The model under review builds one solid part; all positions refer to its coordinate system, in mm. Round coordinates to 2 decimals unless told otherwise and drop trailing zeros. Order: outer loops, then holes, each group sorted by start corner. A loop starts at its lowest first (then second) coordinate and runs counter-clockwise, first axis right, second up. Notation, with made-up numbers: (36, -4.75) -> (68, -4.75) arc R24 cw to (68, 34.25) -> close; hole circle Ø3 at (11, 23). An arc over 180 degrees is marked (long way). Put each result on its own line as item: value. Start each with the question number.
from build123d import *

# Parameters (mm, degrees)
SKETCH_1_W      = 30
SKETCH_1_H      = 60
EXTRUDE_1_DEPTH = 209
SHELL_1_T       = -2


with BuildPart() as part:
    # 草图1 → 凸台-拉伸1 (new, symmetric)
    with BuildSketch(Plane.XY):
        Rectangle(SKETCH_1_W, SKETCH_1_H)
    extrude(amount=EXTRUDE_1_DEPTH, both=True)

    # 抽壳1
    shell_1_openings = [part.faces().sort_by_distance(p)[0] for p in [
        (0, 0, 209),
        (0, 0, -209),
        (0, 30, 0),
    ]]
    offset(amount=SHELL_1_T, openings=shell_1_openings, kind=Kind.INTERSECTION)


solid = part.part
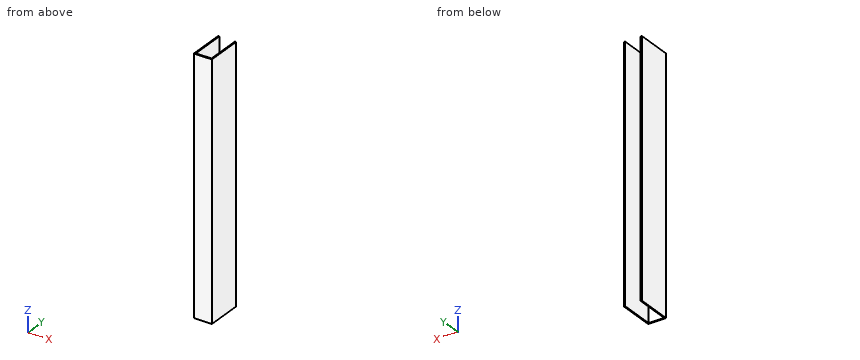
Q1. Take a section at B-B on z = 42.5. Give the boundary of the cut face in (x, y), and give its area (3 significant figures).
Q2. Take a section at A-A on y = -12. Give the boundary of the cut face in (x, z).
Q3. Clearance check with a flat-ended pin moving along its axis: pin 1 Ø1 at (x, z) = (-10, -11) entering from +Y. State where the tip first meets the part, or that it passes through.
Q4. Wall thickness on probe 1 along X at (y, z) = (15.5, -47.5); probe 2 along Y at (x, z) = (-4, 116): over which ranges is each line inside the solid? List them lowest first. Write a range as [from, to].
Q5. Take a section at C-C on x = 4.5. Give the boundary of the cut face in (y, z), and give its area (3 significant figures).
Calculated:
1. outline: (-15, -30) -> (15, -30) -> (15, 30) -> (13, 30) -> (13, -28) -> (-13, -28) -> (-13, 30) -> (-15, 30) -> close
1. area: 292 mm²
2. outline: (-15, -209) -> (-13, -209) -> (-13, 209) -> (-15, 209) -> close; (13, -209) -> (15, -209) -> (15, 209) -> (13, 209) -> close
3. pin 1: stops at y = -28
4. probe 1: x = [-15, -13], [13, 15]
4. probe 2: y = [-30, -28]
5. outline: (-30, -209) -> (-28, -209) -> (-28, 209) -> (-30, 209) -> close
5. area: 836 mm²
